from build123d import *

# Parameters (mm, degrees)
SKETCH1_W           = 20
SKETCH1_H           = 65
SKETCH1_R           = 2.1
SKETCH1_R_2         = 3
SKETCH1_R_3         = 1.6
BOSS_EXTRUDE1_DEPTH = 4


with BuildPart() as part:
    # Sketch1 → Boss-Extrude1 (new body)
    with BuildSketch(Plane.XY):
        Rectangle(SKETCH1_W, SKETCH1_H)
        with Locations((-5, 27.5)):
            Circle(SKETCH1_R, mode=Mode.SUBTRACT)
        with Locations((5, 27.5)):
            Circle(SKETCH1_R, mode=Mode.SUBTRACT)
        with Locations((0, -20.5)):
            Circle(SKETCH1_R_2, mode=Mode.SUBTRACT)
        with Locations((-0.014007289, -12.000011541)):
            Circle(SKETCH1_R_3, mode=Mode.SUBTRACT)
        with Locations((0.014007289, -28.999988459)):
            Circle(SKETCH1_R_3, mode=Mode.SUBTRACT)
    extrude(amount=BOSS_EXTRUDE1_DEPTH)


solid = part.part
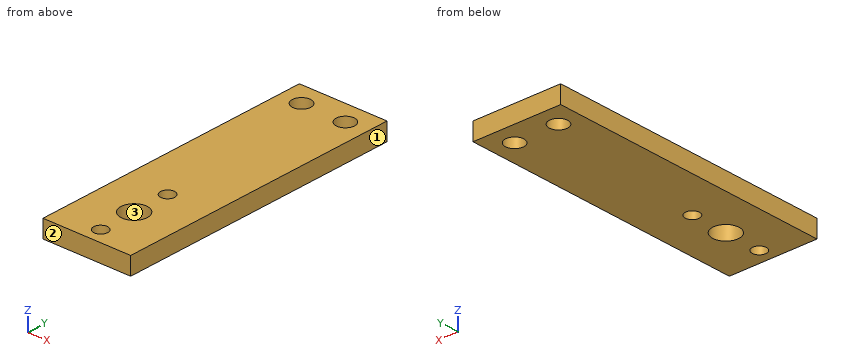
Geometry check sheet. Reference: the model listing, model coordinates, mm. Face numbers are marked on the shaded views. Round coordinates to 2 decimals unless told otherwise and drop trailing zeros. Write each loop counter-clockwise with the first axis right and the second up, starting at its lowest first coordinate (ties: lowest second). Pieces come first, ordered by that corner, then holes. Notation, with made-up numbers: (58, -21) - (65, -21) arc R21 cw to (65, 13) - close; hole circle Ø5 at (-13, 74). An arc over 180 degrees is marked (long way). One line per item, written item: value.
1. Mould release check, pull along Y, two halves, no side actions. Record for the marked faces 1, 2 and 3: released by +Y, released by -Y, zero draft, split by the parting line, or undercut.
The answers:
face 1: zero draft
face 2: released by -Y
face 3: undercut
2. Cross-section at A-A on x = -5. Record the boundary of the cut face in (y, z).
The answers:
outline: (-32.5, 0) - (25.4, 0) - (25.4, 4) - (-32.5, 4) - close; (29.6, 0) - (32.5, 0) - (32.5, 4) - (29.6, 4) - close
3. Scan lines: L1, parallel to Y at x = 0, z = 1.5; L2, parallel to Y at x = -5, z = 2.4; L3, parallel to Y at x = 1.25, z = 0.6. Record each from-to range of solid material in increasing order.
The answers:
L1: y = -32.5 to -30.6, -27.4 to -23.5, -17.5 to -13.6, -10.4 to 32.5
L2: y = -32.5 to 25.4, 29.6 to 32.5
L3: y = -32.5 to -30.02, -27.98 to -23.23, -17.77 to -12.98, -11.02 to 32.5
4. Cross-section at D-D on x = 0. Record the boundary of the cut face in (y, z), and give its area (3 significant figures).
The answers:
outline: (-32.5, 0) - (-30.6, 0) - (-30.6, 4) - (-32.5, 4) - close; (-27.4, 0) - (-23.5, 0) - (-23.5, 4) - (-27.4, 4) - close; (-17.5, 0) - (-13.6, 0) - (-13.6, 4) - (-17.5, 4) - close; (-10.4, 0) - (32.5, 0) - (32.5, 4) - (-10.4, 4) - close
area: 210 mm^2
5. Cross-section at B-B on y = 27.5. Record the boundary of the cut face in (x, z).
The answers:
outline: (-10, 0) - (-7.1, 0) - (-7.1, 4) - (-10, 4) - close; (-2.9, 0) - (2.9, 0) - (2.9, 4) - (-2.9, 4) - close; (7.1, 0) - (10, 0) - (10, 4) - (7.1, 4) - close
6. Cross-section at C-C on y = -20.5. Record the boundary of the cut face in (x, z).
The answers:
outline: (-10, 0) - (-3, 0) - (-3, 4) - (-10, 4) - close; (3, 0) - (10, 0) - (10, 4) - (3, 4) - close
